Part model, mm, in its own coordinate system. A direction names the side the tool comes from. Round coordinates to 2 decimals unless told otherwise and drop trailing zeros. Write each loop counter-clockwise with the first axis right and the second up, starting at its lowest first coordinate (ties: lowest second). Pieces come first, ordered by that corner, then holes. Notation, with made-up numbers: (-36, 53.25) -> (2, 53.25) arc R12 ccw to (2, 63.25) -> close; hole circle Ø6 at (-29, 26). An arc over 180 degrees is marked (long way). Use CSV: the item, a comma, the result in double quotes. Start each with the question number.
(1) Saw through at A-A (z = 9). Give the cut face in (x, y).
(2) Probe line 1 (X direction, y = 12.35, z = 37.8); line 2 (X direction, y = 1.25, z = 37.8); line 3 (Z direction, x = 68.8, y = 11.65). List the from-to ranges inside material, lowest first. Write a range as [from, to].
(3) Two-plate mould, pull along Z, no slides. Class faces 1 (the flat face through (41, 15, 32)), 2 (the flat face through (58, 12.9, 51)), 3 (the flat face through (41, 8, 0)): released by +Z, released by -Z, zero draft, split by the parting line, or undercut.
(4) Saw through at D-D (x = 56.5). Give the cut face in (y, z).
(5) Saw through at C-C (y = 3.25). Give the cut face in (x, z), plus the area to 3 significant figures.
(6) Drop a flat-ended pin along its axis: pin 1 (9 mm diameter, centred on x = 68.8, z = 37.8, fed in from +Y). Give the stop position or say it passes through.
(7) Saw through at B-B (x = 68.8). Give the cut face in (y, z), plus the area to 3 significant figures.
(8) Which spindle directions (+Z, -Z, +X, -X, +Y, -Y) get a long thin tool onto all of the face, cutting with end or side? Do faces 4 (the cylindrical face through (69.85, 0.79, 34.46)), 5 (the flat face through (41, 8, 64)), 6 (the cylindrical face through (27.852, 13.965, 53.292)). Say none if no direction does.
```python
from build123d import *

# Parameters (mm, degrees)
SKETCH1_W                                            = 83
SKETCH1_H                                            = 15
BOSS_EXTRUDE1_DEPTH                                  = 64
HOLE_SIZE_PER_SOCKET_HEAD_CAP_SCREW_TYPE_D           = 5.5
HOLE_SIZE_PER_SOCKET_HEAD_CAP_SCREW_TYPE_CBORE_D     = 10
HOLE_SIZE_PER_SOCKET_HEAD_CAP_SCREW_TYPE_CBORE_DEPTH = 6
SKETCH5_R                                            = 3.5
CUT_EXTRUDE1_DEPTH                                   = 1.6
M5_TAPPED_HOLE1_D                                    = 4.2
SKETCH8_R                                            = 4.5
CUT_EXTRUDE2_DEPTH                                   = 2.1


with BuildPart() as part:
    # Sketch1 → Boss-Extrude1 (new body)
    with BuildSketch(Plane.XY):
        with Locations((41.5, 7.5)):
            Rectangle(SKETCH1_W, SKETCH1_H)
    extrude(amount=BOSS_EXTRUDE1_DEPTH)

    # Hole size per socket head cap screw type 1 (through all)
    with Locations(Plane(origin=(0, 15, 0), x_dir=(1, 0, 0), z_dir=(0, 1, 0))):
        with Locations((18.8, -37.8), (68.8, -37.8)):
            CounterBoreHole(HOLE_SIZE_PER_SOCKET_HEAD_CAP_SCREW_TYPE_D / 2, HOLE_SIZE_PER_SOCKET_HEAD_CAP_SCREW_TYPE_CBORE_D / 2, HOLE_SIZE_PER_SOCKET_HEAD_CAP_SCREW_TYPE_CBORE_DEPTH)

    # Sketch5 → Cut-Extrude1 (cut)
    with BuildSketch(Plane.XZ):
        with Locations(Location((18.8, 37.8, 0), (0, 0, 270))):
            Circle(SKETCH5_R)
        with Locations(Location((68.8, 37.8, 0), (0, 0, 270))):
            Circle(SKETCH5_R)
    extrude(amount=-CUT_EXTRUDE1_DEPTH, mode=Mode.SUBTRACT)

    # M5 Tapped Hole1 (through all)
    with Locations(Plane(origin=(0, 15, 0), x_dir=(1, 0, 0), z_dir=(0, 1, 0))):
        with Locations((56.5, -9), (26.5, -9), (26.5, -49), (56.5, -49)):
            Hole(M5_TAPPED_HOLE1_D / 2)

    # Sketch8 → Cut-Extrude2 (cut)
    with BuildSketch(Plane(origin=(0, 15, 0), x_dir=(1, 0, 0), z_dir=(0, 1, 0))):
        with Locations(Location((26.5, -49, 0), (0, 0, 270))):
            Circle(SKETCH8_R)
        with Locations(Location((56.5, -49, 0), (0, 0, 270))):
            Circle(SKETCH8_R)
    extrude(amount=-CUT_EXTRUDE2_DEPTH, mode=Mode.SUBTRACT)


solid = part.part
```
Answers:
1,outline,"(0, 0) -> (24.4, 0) -> (24.4, 15) -> (0, 15) -> close; (28.6, 0) -> (54.4, 0) -> (54.4, 15) -> (28.6, 15) -> close; (58.6, 0) -> (83, 0) -> (83, 15) -> (58.6, 15) -> close"
2,line 1,"x = [0, 13.8], [23.8, 63.8], [73.8, 83]"
2,line 2,"x = [0, 15.3], [22.3, 65.3], [72.3, 83]"
2,line 3,"z = [0, 32.8], [42.8, 64]"
3,face 1,"zero draft"
3,face 2,"undercut"
3,face 3,"released by -Z"
4,outline,"(0, 0) -> (15, 0) -> (15, 6.9) -> (0, 6.9) -> close; (0, 11.1) -> (15, 11.1) -> (15, 44.5) -> (12.9, 44.5) -> (12.9, 46.9) -> (0, 46.9) -> close; (0, 51.1) -> (12.9, 51.1) -> (12.9, 53.5) -> (15, 53.5) -> (15, 64) -> (0, 64) -> close"
5,outline,"(0, 0) -> (83, 0) -> (83, 64) -> (0, 64) -> close; hole circle Ø5.5 at (18.8, 37.8); hole circle Ø4.2 at (26.5, 9); hole circle Ø4.2 at (26.5, 49); hole circle Ø4.2 at (56.5, 9); hole circle Ø4.2 at (56.5, 49); hole circle Ø5.5 at (68.8, 37.8)"
5,area,"5,210 mm²"
6,pin 1,"stops at y = 9"
7,outline,"(0, 0) -> (15, 0) -> (15, 32.8) -> (9, 32.8) -> (9, 35.05) -> (1.6, 35.05) -> (1.6, 34.3) -> (0, 34.3) -> close; (0, 41.3) -> (1.6, 41.3) -> (1.6, 40.55) -> (9, 40.55) -> (9, 42.8) -> (15, 42.8) -> (15, 64) -> (0, 64) -> close"
7,area,"848 mm²"
8,face 4,"-Y"
8,face 5,"+Z, +X, -X, +Y, -Y"
8,face 6,"+Y"
